Check sheet for the modelled part. Datum: model origin and axes. Units: mm. Round coordinates to 2 decimals unless told otherwise and drop trailing zeros. Write each loop counter-clockwise with the first axis right and the second up, starting at its lowest first coordinate (ties: lowest second). Pieces come first, ordered by that corner, then holes.
Item 1: Cross-section at B-B on y = -11.5. Enter the section's corners in (x, z).
Item 2: Go/stop test with flat-tipped pins: pin 1 Ø7.5 at (x, y) = (10, 2.5) entering from +Z; pin 2 Ø5.5 at (x, y) = (-150, 0) entering from -Z. Record where each tip stops, or that it passes through.
Item 3: Material ranges on line 1 (X direction, y = -0.75, z = -4.25); line 2 (Y direction, x = 10, z = 1.5); line 3 (Y direction, x = 170, z = 0.75), recorded low to high.
Item 4: Cross-section at C-C on x = 170. Enter the section's corners in (y, z).
Item 5: Cross-section at A-A on x = -150. Enter the section's corners in (y, z).
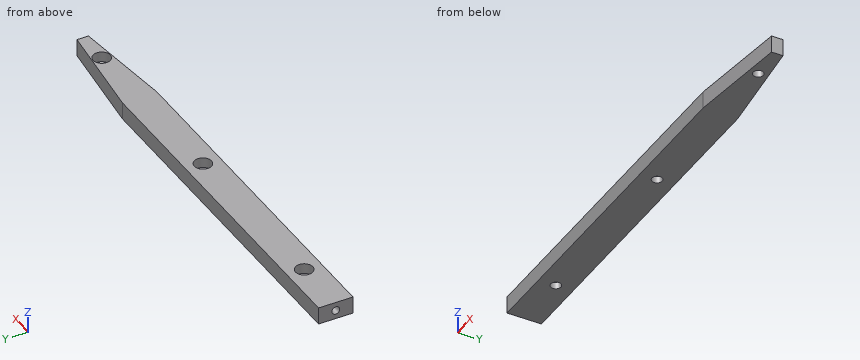
from build123d import *

# Parameters (mm, degrees)
EXTRUDE_1_DEPTH           = 7.5
HOLE_WIZARD_M8_1_D        = 6.8
HOLE_WIZARD_M8_1_DEPTH    = 19.75
HOLE_WIZARD_M8_1_TIP      = 2.042926105
HOLE_WIZARD_1_D           = 9
HOLE_WIZARD_1_CBORE_D     = 15
HOLE_WIZARD_1_CBORE_DEPTH = 9


with BuildPart() as part:
    # 草图1 → 凸台-拉伸1 (new, symmetric)
    with BuildSketch(Plane.XY):
        Polygon((200, 5), (110, 15), (-200, 15), (-200, -15), (110, -15), (200, -5), align=None)
    extrude(amount=EXTRUDE_1_DEPTH, both=True)

    # M8 螺纹孔1
    with Locations(Plane(origin=(-200, 0, 0), x_dir=(0, 0, -1), z_dir=(-1, 0, 0))):
        with Locations((0, 0)):
            Hole(HOLE_WIZARD_M8_1_D / 2, depth=HOLE_WIZARD_M8_1_DEPTH)
            with Locations((0, 0, -(HOLE_WIZARD_M8_1_DEPTH + HOLE_WIZARD_M8_1_TIP / 2))):  # 118° drill point
                Cone(0, HOLE_WIZARD_M8_1_D / 2, HOLE_WIZARD_M8_1_TIP, mode=Mode.SUBTRACT)

    # 打孔尺寸(%根据)内六角圆柱头螺钉的类型1 (through all)
    with Locations(Plane(origin=(-150, 0, 7.5), x_dir=(1, 0, 0), z_dir=(0, 0, 1))):
        with Locations((0, 0), (320, 0), (160, 0)):
            CounterBoreHole(HOLE_WIZARD_1_D / 2, HOLE_WIZARD_1_CBORE_D / 2, HOLE_WIZARD_1_CBORE_DEPTH)


solid = part.part
Response values:
1. outline: (-200, -7.5) - (141.5, -7.5) - (141.5, 7.5) - (-200, 7.5) - close
2. pin 1: stops at z = -1.5
2. pin 2: passes through
3. line 1: x = -200 to -154.44, -145.56 to 5.56, 14.44 to 165.56, 174.44 to 200
3. line 2: y = -15 to -7.5, 7.5 to 15
3. line 3: y = -8.33 to -7.5, 7.5 to 8.33
4. outline: (-8.33, -7.5) - (-4.5, -7.5) - (-4.5, -1.5) - (-7.5, -1.5) - (-7.5, 7.5) - (-8.33, 7.5) - close; (4.5, -7.5) - (8.33, -7.5) - (8.33, 7.5) - (7.5, 7.5) - (7.5, -1.5) - (4.5, -1.5) - close
5. outline: (-15, -7.5) - (-4.5, -7.5) - (-4.5, -1.5) - (-7.5, -1.5) - (-7.5, 7.5) - (-15, 7.5) - close; (4.5, -7.5) - (15, -7.5) - (15, 7.5) - (7.5, 7.5) - (7.5, -1.5) - (4.5, -1.5) - close
